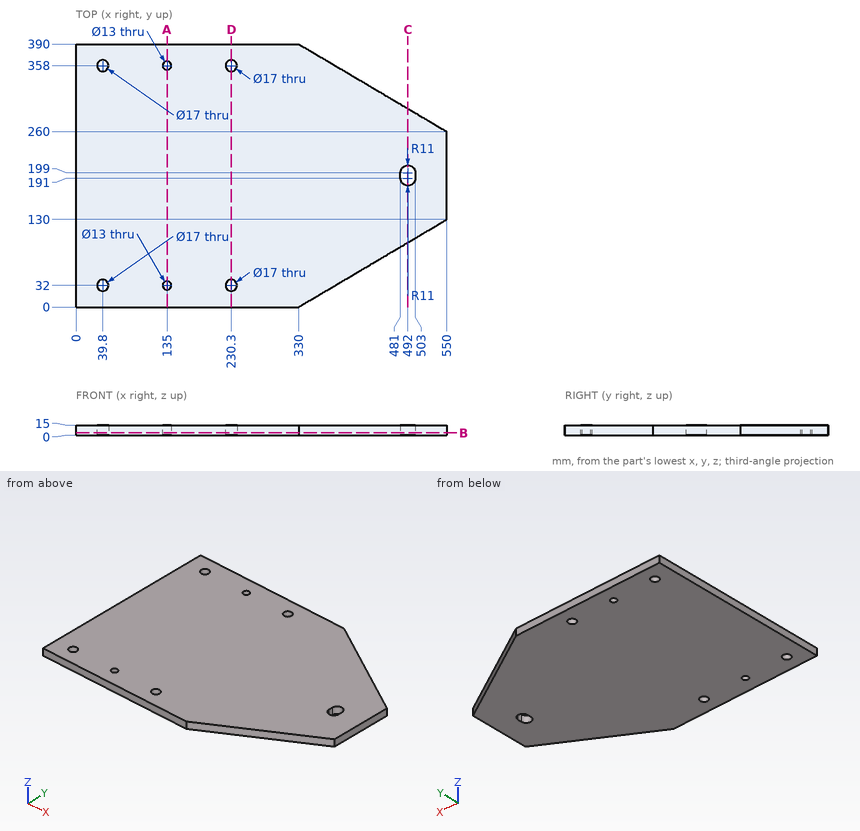
Answer from the drawing. Dimensions are ordinates in mm from the lowest x, y and z of the part. Coordinates: 2 decimals unless noted, no trailing zeros. Write each loop counter-clockwise with the first axis right and the second up, starting at its lowest first coordinate (ties: lowest second). Pieces come first, ordered by that corner, then holes. Notation, with made-up numbers: M -38.75,-20 L 10.25,-20 A37 cw 10.25,18 Z; hole C 61.25,73 d11. An arc over 180 degrees is marked long. Use one line per item in the form item = value. Start each with the question number.
1. The part is cut by section B-B (z = 3.25). Give the vertices of the cut face in (x, y), plus the area to 3 significant figures.
2. The part is cut by section C-C (x = 492). Give the vertices of the cut face in (y, z).
3. The part is cut by section D-D (x = 230.3). Give the vertices of the cut face in (y, z).
4. Straight lines are drawn through the part: probe 1 along Y at (x, z) = (135, 7.25); probe 2 along Y at (x, z) = (39.8, 9.75); probe 3 along X at (y, z) = (358, 9.5). For each, find the intervals that lie inside material, in ascending order. Write a range as from..to.
5. The part is cut by section A-A (x = 135). Give the vertices of the cut face in (y, z), plus the area to 3 significant figures.
6. Each of these flat-tipped pins is pushed along its axis until it touches: P1, Ø15.5, axis at x = 230.3, y = 358, coming from the +Z side (3 decimals); P2, Ø3, axis at x = 438.5, z = 8.5, coming from the +Y side; P3, Ø5, axis at x = 340, z = 4, coming from the -Y side. Where does it stop, or does it pass through?
Evaluation:
q1.outline = M 0,0 L 330,0 L 550,130 L 550,260 L 330,390 L 0,390 Z; hole C 39.8,32 d17; hole C 39.8,358 d17; hole C 135,32 d13; hole C 135,358 d13; hole C 230.3,32 d17; hole C 230.3,358 d17; hole M 481,191 A11 ccw 503,191 L 503,199 A11 ccw 481,199 Z
q1.area = 184,000 mm^2
q2.outline = M 95.73,0 L 180,0 L 180,15 L 95.73,15 Z; M 210,0 L 294.27,0 L 294.27,15 L 210,15 Z
q3.outline = M 0,0 L 23.5,0 L 23.5,15 L 0,15 Z; M 40.5,0 L 349.5,0 L 349.5,15 L 40.5,15 Z; M 366.5,0 L 390,0 L 390,15 L 366.5,15 Z
q4.probe_1 = 0..25.5, 38.5..351.5, 364.5..390
q4.probe_2 = 0..23.5, 40.5..349.5, 366.5..390
q4.probe_3 = 0..31.3, 48.3..128.5, 141.5..221.8, 238.8..384.15
q5.outline = M 0,0 L 25.5,0 L 25.5,15 L 0,15 Z; M 38.5,0 L 351.5,0 L 351.5,15 L 38.5,15 Z; M 364.5,0 L 390,0 L 390,15 L 364.5,15 Z
q5.area = 5,460 mm^2
q6.P1 = through
q6.P2 = 326.77
q6.P3 = 4.43
